Check sheet for the modelled part. Datum: model origin and axes. Units: mm. Face numbers are marked on the shaded views. A direction names the side the tool comes from. Round coordinates to 2 decimals unless told otherwise and drop trailing zeros. Write each loop counter-clockwise with the first axis right and the second up, starting at its lowest first coordinate (ties: lowest second). Pieces come first, ordered by that corner, then holes.
Item 1: Depth check by flat-ended pin: pin 1 (2.5 mm diameter, centred on x = -5, y = -34.25, fed in from +Z); pin 2 (0.9 mm diameter, centred on x = 7, z = 6.5, fed in from +Y); pin 3 (5 mm diameter, centred on x = 10.5, y = -19, fed in from -Z); pin 4 (6 mm diameter, centred on x = -5, y = 14.24, fed in from -Z). Enter the tip coordinate at first touch or a pass-through.
Item 2: Section check D-D, the plane y = -3. Record the cut outline in (x, z), plus the area to 3 significant figures.
Item 3: Section check C-C, the plane z = 8.5. Record the cut outline in (x, y), plus the area to 3 significant figures.
Item 4: Material ranges on line 1 along X through (y, z) = (-34.25, -26.4); line 2 along X through (y, z) = (-22, 14); line 3 along X through (y, z) = (-12.5, -12.5), recorded low to high.
Item 5: Set-up check for the marked faces 1, 2 and 3: record each of +Z, -Z, +X, -X, +Y, -Y from which the full face is reachable in a straight line by a thin tool's end or side.
Item 6: Section check A-A, the plane x = -5. Record the cut outline in (y, z), plus the area to 3 significant figures.
Item 7: Release check for a two-part mould opening along X. For the marked faces 4, 5 and 6 record: pulls with the +X half, pulls with the -X half, needs draft (parallel to the pull), parting line crosses it, or undercut.
Item 8: Section check B-B, the plane x = -1.75. Record the cut outline in (y, z), plus the area to 3 significant figures.
from build123d import *

# Parameters (mm, degrees)
SKETCH2_W           = 21
SKETCH2_H           = 40.5
BOSS_EXTRUDE1_DEPTH = 2.5
SKETCH3_W           = 3
SKETCH3_H           = 33
BOSS_EXTRUDE2_DEPTH = 14
SKETCH4_R           = 10
CUT_EXTRUDE1_DEPTH  = 40.501767279
BOSS_EXTRUDE3_DEPTH = 20.25
FILLET1_R           = 3
FILLET2_R           = 2.5
BOSS_EXTRUDE4_DEPTH = 2.5
SKETCH7_R           = 2
CUT_EXTRUDE2_DEPTH  = 56.162442887
BOSS_EXTRUDE5_DEPTH = 21
SKETCH10_R          = 2.25
CUT_EXTRUDE3_DEPTH  = 21


with BuildPart() as part:
    # Sketch2 → Boss-Extrude1 (new body)
    with BuildSketch(Plane.XY):
        with Locations((0.095633845, -10.004131531)):
            Rectangle(SKETCH2_W, SKETCH2_H)
    extrude(amount=BOSS_EXTRUDE1_DEPTH)

    # Sketch3 → Boss-Extrude2 (add)
    with BuildSketch(Plane.XY.offset(2.5)):
        with Locations((-7.404366155, -10.004131531)):
            Rectangle(SKETCH3_W, SKETCH3_H)
        with Locations((7.404366155, -10.004131531)):
            Rectangle(SKETCH3_W, SKETCH3_H)
    extrude(amount=BOSS_EXTRUDE2_DEPTH)

    # Sketch4 → Cut-Extrude1 (cut, through all)
    with BuildSketch(Plane(origin=(8.904366155, 0, 0), x_dir=(0, 0, -1), z_dir=(1, 0, 0))):
        with Locations((-16.5, -10.004131531)):
            Circle(SKETCH4_R)
    extrude(amount=-CUT_EXTRUDE1_DEPTH, mode=Mode.SUBTRACT)

    # Sketch5 → Boss-Extrude3 (add, symmetric)
    with BuildSketch(Plane(origin=(0, -10.004131531, 0), x_dir=(1, 0, 0), z_dir=(0, 1, 0))):
        Polygon((10.595633845, 0), (10.595633845, 29.5), (13.095633845, 29.5), (13.095633845, -2.5), (10.595633845, -2.5), align=None)
    extrude(amount=BOSS_EXTRUDE3_DEPTH, both=True)

    # Fillet1
    fillet1_edges = [part.edges().sort_by_distance(p)[0] for p in [
        (13.095633845, -10.004131531, 2.5),
    ]]
    fillet(fillet1_edges, radius=FILLET1_R)

    # Fillet2
    fillet2_edges = [part.edges().sort_by_distance(p)[0] for p in [
        (10.595633845, -10.004131531, 0),
    ]]
    fillet(fillet2_edges, radius=FILLET2_R)

    # Sketch6 → Boss-Extrude4 (add)
    with BuildSketch(Plane(origin=(13.095633845, 0, 0), x_dir=(0, 0, -1), z_dir=(1, 0, 0))):
        with BuildLine():
            Line((29.5, -30.254131531), (29.5, -36.254131531))
            ThreePointArc((29.5, -36.254131531), (28.328427125, -39.082558656), (25.5, -40.254131531))
            Line((25.5, -40.254131531), (7.39536549, -40.254131531))
            ThreePointArc((7.39536549, -40.254131531), (4.566938365, -39.082558656), (3.39536549, -36.254131531))
            Line((3.39536549, -36.254131531), (3.39536549, -30.254131531))
            Line((3.39536549, -30.254131531), (29.5, -30.254131531))
        make_face()
        with BuildLine():
            Line((3.39536549, 10.245868469), (29.5, 10.245868469))
            Line((29.5, 10.245868469), (29.5, 16.245868469))
            ThreePointArc((29.5, 16.245868469), (28.328427125, 19.074295594), (25.5, 20.245868469))
            Line((25.5, 20.245868469), (7.39536549, 20.245868469))
            ThreePointArc((7.39536549, 20.245868469), (4.566938365, 19.074295594), (3.39536549, 16.245868469))
            Line((3.39536549, 16.245868469), (3.39536549, 10.245868469))
        make_face()
    extrude(amount=-BOSS_EXTRUDE4_DEPTH)

    # Sketch7 → Cut-Extrude2 (cut, through all)
    with BuildSketch(Plane(origin=(13.095633845, 0, 0), x_dir=(0, 0, -1), z_dir=(1, 0, 0))):
        with Locations((21.39536549, -34.254131531)):
            Circle(SKETCH7_R)
        with Locations((10.39536549, -34.254131531)):
            Circle(SKETCH7_R)
        with Locations((10.39536549, 14.245868469)):
            Circle(SKETCH7_R)
        with Locations((21.39536549, 14.245868469)):
            Circle(SKETCH7_R)
    extrude(amount=-CUT_EXTRUDE2_DEPTH, mode=Mode.SUBTRACT)

    # Sketch9 → Boss-Extrude5 (add)
    with BuildSketch(Plane.ZY.offset(-10.595633845)):
        with BuildLine():
            Line((-28.328427125, -39.082558656), (-28.328427125, -29.914909502))
            Line((-28.328427125, -29.914909502), (-25.5, -29.914909502))
            Line((-25.5, -29.914909502), (-25.5, -40.254131531))
            ThreePointArc((-25.5, -40.254131531), (-27.030733729, -39.949649661), (-28.328427125, -39.082558656))
        make_face()
    boss_extrude5 = extrude(amount=BOSS_EXTRUDE5_DEPTH)

    # Mirror1: Boss-Extrude5 across plane
    add(boss_extrude5.mirror(Plane.ZX.offset(-10.004131531)))

    # Sketch10 → Cut-Extrude3 (cut)
    with BuildSketch(Plane(origin=(0, 0, -28.328427125), x_dir=(-1, 0, 0), z_dir=(0, 0, -1))):
        with Locations(Location((-5, -34.25, 0), (0, 0, 90))):
            Circle(SKETCH10_R)
        with Locations(Location((5, -34.25, 0), (0, 0, 90))):
            Circle(SKETCH10_R)
    cut_extrude3 = extrude(amount=-CUT_EXTRUDE3_DEPTH, mode=Mode.SUBTRACT)

    # Mirror2: Cut-Extrude3 across plane
    add(cut_extrude3.mirror(Plane.ZX.offset(-10.004131531)), mode=Mode.SUBTRACT)


solid = part.part
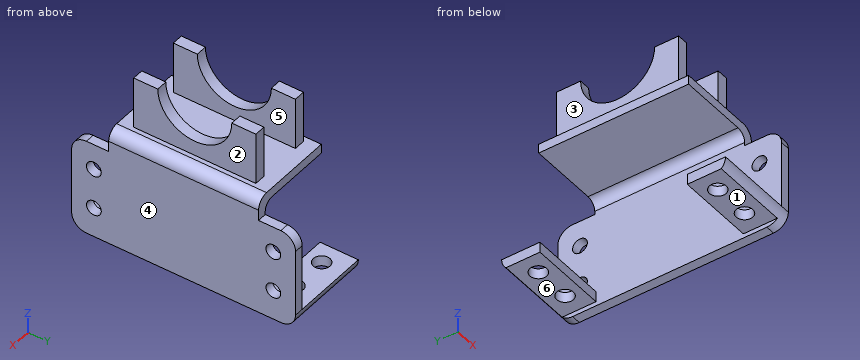
Values found:
1. pin 1: passes through
1. pin 2: stops at y = 6.5
1. pin 3: stops at z = -29.5
1. pin 4: stops at z = -28.33
2. outline: (-10.4, 0) - (8.1, 0) arc R2.5 cw to (10.6, -2.5) - (10.6, -29.5) - (13.1, -29.5) - (13.1, -0.5) arc R3 ccw to (10.1, 2.5) - (8.9, 2.5) - (8.9, 9.36) - (5.9, 9.36) - (5.9, 2.5) - (-5.9, 2.5) - (-5.9, 9.36) - (-8.9, 9.36) - (-8.9, 2.5) - (-10.4, 2.5) - close
2. area: 173 mm2
3. outline: (-8.9, -26.5) - (-5.9, -26.5) - (-5.9, -16) - (-8.9, -16) - close; (-8.9, -4) - (-5.9, -4) - (-5.9, 6.5) - (-8.9, 6.5) - close; (5.9, -26.5) - (8.9, -26.5) - (8.9, -16) - (5.9, -16) - close; (5.9, -4) - (8.9, -4) - (8.9, 6.5) - (5.9, 6.5) - close
3. area: 126 mm2
4. line 1: x = -10.4 to -7.25, -2.75 to 2.75, 7.25 to 13.1
4. line 2: x = -8.9 to -5.9, 5.9 to 8.9
4. line 3: x = 10.6 to 13.1
5. face 1: -Z, -X, +Y, -Y
5. face 2: +Z, +X, +Y, -Y
5. face 3: +Z, -X, +Y, -Y
6. outline: (-40.25, -25.5) arc R4 ccw to (-39.08, -28.33) - (-36.5, -28.33) - (-36.5, -25.5) - close; (-32, -28.33) - (-29.91, -28.33) - (-29.91, -25.5) - (-32, -25.5) - close; (-30.25, 0) - (10.25, 0) - (10.25, 2.5) - (-30.25, 2.5) - close; (9.91, -28.33) - (11.99, -28.33) - (11.99, -25.5) - (9.91, -25.5) - close; (16.49, -28.33) - (19.07, -28.33) arc R4 ccw to (20.25, -25.5) - (16.49, -25.5) - close
6. area: 132 mm2
7. face 4: pulls with the +X half
7. face 5: undercut
7. face 6: needs draft
8. outline: (-40.25, -25.5) arc R4 ccw to (-39.08, -28.33) - (-29.91, -28.33) - (-29.91, -25.5) - close; (-30.25, 0) - (10.25, 0) - (10.25, 2.5) - (-30.25, 2.5) - close; (9.91, -28.33) - (19.07, -28.33) arc R4 ccw to (20.25, -25.5) - (9.91, -25.5) - close
8. area: 158 mm2
